```python
from build123d import *

# Parameters (mm, degrees)
SKETCH1_R           = 12
BOSS_EXTRUDE1_DEPTH = 2
SKETCH2_R           = 15.5
SKETCH2_R_2         = 0.7
BOSS_EXTRUDE2_DEPTH = 1.5
SKETCH3_R           = 10.15
CUT_EXTRUDE1_DEPTH  = 1
FILLET1_R           = 1.2
SKETCH4_R           = 1.25
CUT_EXTRUDE2_DEPTH  = 0.5
SKETCH5_R           = 5
CUT_EXTRUDE3_DEPTH  = 23.19797288
CHAMFER1_SIZE       = 0.5
CUT_EXTRUDE4_DEPTH  = 1


with BuildPart() as part:
    # Sketch1 → Boss-Extrude1 (new body)
    with BuildSketch(Plane.XY):
        Circle(SKETCH1_R)
    extrude(amount=BOSS_EXTRUDE1_DEPTH)

    # Sketch2 → Boss-Extrude2 (add)
    with BuildSketch(Plane.XY.offset(2)):
        Circle(SKETCH2_R)
        with Locations((0, 13.25)):
            Circle(SKETCH2_R_2, mode=Mode.SUBTRACT)
        with Locations((13.25, 0)):
            Circle(SKETCH2_R_2, mode=Mode.SUBTRACT)
        with Locations((0, -13.25)):
            Circle(SKETCH2_R_2, mode=Mode.SUBTRACT)
        with Locations((-13.25, 0)):
            Circle(SKETCH2_R_2, mode=Mode.SUBTRACT)
    extrude(amount=BOSS_EXTRUDE2_DEPTH)

    # Sketch3 → Cut-Extrude1 (cut)
    with BuildSketch(Plane.XY.offset(3.5)):
        Circle(SKETCH3_R)
    extrude(amount=-CUT_EXTRUDE1_DEPTH, mode=Mode.SUBTRACT)

    # Fillet1
    fillet1_edges = [part.edges().sort_by_distance(p)[0] for p in [
        (-12, 0, 0),
    ]]
    fillet(fillet1_edges, radius=FILLET1_R)

    # Sketch4 → Cut-Extrude2 (cut)
    with BuildSketch(Plane(origin=(0, 0, 2), x_dir=(-1, 0, 0), z_dir=(0, 0, -1))):
        with Locations((0, 13.25)):
            Circle(SKETCH4_R)
        with Locations((13.25, 0)):
            Circle(SKETCH4_R)
        with Locations((0, -13.25)):
            Circle(SKETCH4_R)
        with Locations((-13.25, 0)):
            Circle(SKETCH4_R)
    extrude(amount=-CUT_EXTRUDE2_DEPTH, mode=Mode.SUBTRACT)

    # Sketch5 → Cut-Extrude3 (cut, through all)
    with BuildSketch(Plane(origin=(0, 0, 0), x_dir=(-1, 0, 0), z_dir=(0, 0, -1))):
        Circle(SKETCH5_R)
    extrude(amount=-CUT_EXTRUDE3_DEPTH, mode=Mode.SUBTRACT)

    # Chamfer1
    chamfer1_edges = [part.edges().sort_by_distance(p)[0] for p in [
        (5, 0, 2.5),
        (5, 0, 0),
    ]]
    chamfer(chamfer1_edges, length=CHAMFER1_SIZE)

    # Sketch6 → Cut-Extrude4 (cut)
    with BuildSketch(Plane.XY.offset(3.5)):
        Polygon((-0.707106781, 0.707106781), (0.707106781, -0.707106781), (-10.253048327, -11.66726189), (-11.66726189, -10.253048327), align=None)
    extrude(amount=-CUT_EXTRUDE4_DEPTH, mode=Mode.SUBTRACT)


solid = part.part
```
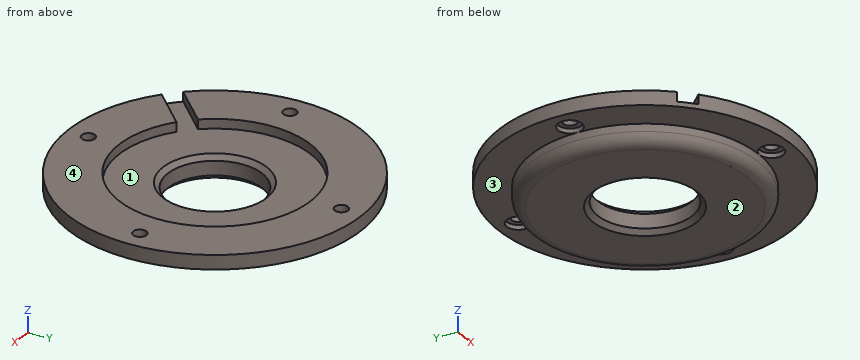
Source: CAD feature listing. Evaluate the final solid. Frame: model axes, mm. Face numbers are marked on the shaded views. A direction names the side the tool comes from. Give positions to 0.01 mm unless a question says otherwise; leave off trailing zeros. Write each loop counter-clockwise with the first axis right and the second up, starting at its lowest first coordinate (ties: lowest second). Pieces come first, ordered by that corner, then holes. Notation, with made-up numbers: (-13.5, 24.5) - (6.5, 24.5) arc R10 ccw to (6.5, 28.5) - close; hole circle Ø9 at (-23, -21.75). An arc over 180 degrees is marked (long way). One line per item, written item: value. Start each with the question number.
Q1. Section query B-B, the plane y = -13.25. Return the cut outline in (x, z), then the cut area to 3 significant figures.
Q2. Section query A-A, the plane z = 2.95. Return the cut outline in (x, y).
Q3. First-contact query: pin 1 Ø1.2 at (x, y) = (0, -13.5) entering from -Z; pin 2 Ø2 at (x, y) = (0.5, 13.5) entering from -Z; pin 3 Ø2 at (y, z) = (-3.5, 2.5) entering from +X. Flat tips, straight axial feed; report the tip coordinate or a pass-through.
Q4. Set-up query: the marked faces 3 and 4. Return all of +Z, -Z, +X, -X, +Y, -Y with unobstructed straight access to the full face (end or side cutting, diameter ignored); none if empty.
Q5. Draft query along X for the marked faces 1 and 2. Return one class per face: +X half, -X half, draft (parallel to the pull), parting line (faces both ways), or undercut.
Q6. Material intervals for probe 1 along X at (y, z) = (0, 2.9); probe 2 along Z at (x, y) = (-7.5, -4), sorted ascending. Write a range as from..to.
Answer:
1. outline: (-8.04, 2) - (-1.25, 2) - (-1.25, 2.5) - (-0.7, 2.5) - (-0.7, 3.5) - (-8.04, 3.5) - close; (0.7, 2.5) - (1.25, 2.5) - (1.25, 2) - (8.04, 2) - (8.04, 3.5) - (0.7, 3.5) - close
1. area: 21.5 mm2
2. outline: (-11.64, -10.23) - (-7.85, -6.44) arc R10.15 cw (long way) to (-6.44, -7.85) - (-10.23, -11.64) arc R15.5 ccw (long way) to start; hole circle Ø1.4 at (-13.25, 0); hole circle Ø1.4 at (0, -13.25); hole circle Ø1.4 at (0, 13.25); hole circle Ø1.4 at (13.25, 0)
3. pin 1: stops at z = 2.5
3. pin 2: stops at z = 2
3. pin 3: stops at x = 15.3
4. face 3: -Z
4. face 4: +Z, +X, -X, +Y, -Y
5. face 1: undercut
5. face 2: draft
6. probe 1: x = -15.5..-13.95, -12.55..-10.15, 10.15..12.55, 13.95..15.5
6. probe 2: z = 0..2.5
